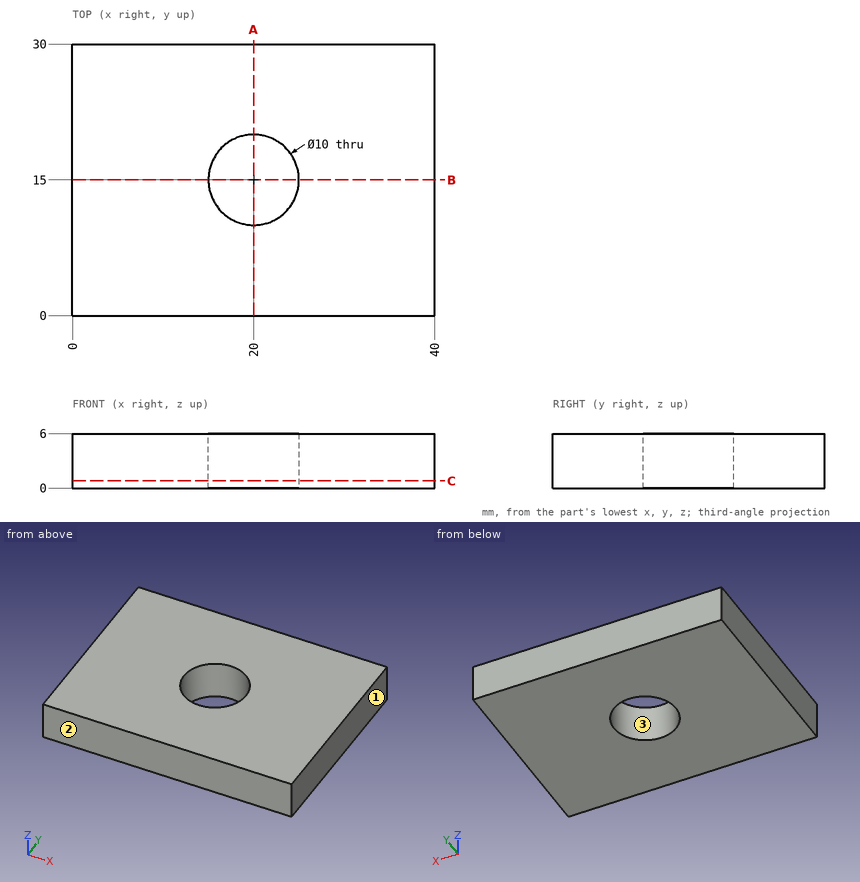
Drawing for the job (mm, zero at the part's lowest x, y, z). Round coordinates to 2 decimals unless told otherwise and drop trailing zeros. Loops run counter-clockwise (first coordinate to the right, second up) from the corner with the lowest first, then second, coordinate; pieces in that order, holes last.
1. Band-saw the part on C-C, the plane z = 0.8. List the corners of the cut face in (x, y), and give its area (3 significant figures).
Check values:
outline: (0, 0) - (40, 0) - (40, 30) - (0, 30) - close; hole circle Ø10 at (20, 15)
area: 1,120 mm2
2. Mould opens along X. For the marked faces 1, 2 and 3 say: +X half, -X half, draft (parallel to the pull), parting line (faces both ways), or undercut.
Check values:
face 1: +X half
face 2: draft
face 3: undercut
3. Band-saw the part on B-B, the plane y = 15. List the corners of the cut face in (x, z), and give its area (3 significant figures).
Check values:
outline: (0, 0) - (15, 0) - (15, 6) - (0, 6) - close; (25, 0) - (40, 0) - (40, 6) - (25, 6) - close
area: 180 mm2
4. Band-saw the part on A-A, the plane x = 20. List the corners of the cut face in (y, z).
Check values:
outline: (0, 0) - (10, 0) - (10, 6) - (0, 6) - close; (20, 0) - (30, 0) - (30, 6) - (20, 6) - close
5. Wall check: probe 1 along Y at (x, z) = (20, 1.8); probe 2 along X at (y, z) = (16.5, 5.35); probe 3 along Y at (x, z) = (23, 5). Give the ranges that are in metal, low to high.
Check values:
probe 1: y = 0 to 10, 20 to 30
probe 2: x = 0 to 15.23, 24.77 to 40
probe 3: y = 0 to 11, 19 to 30
